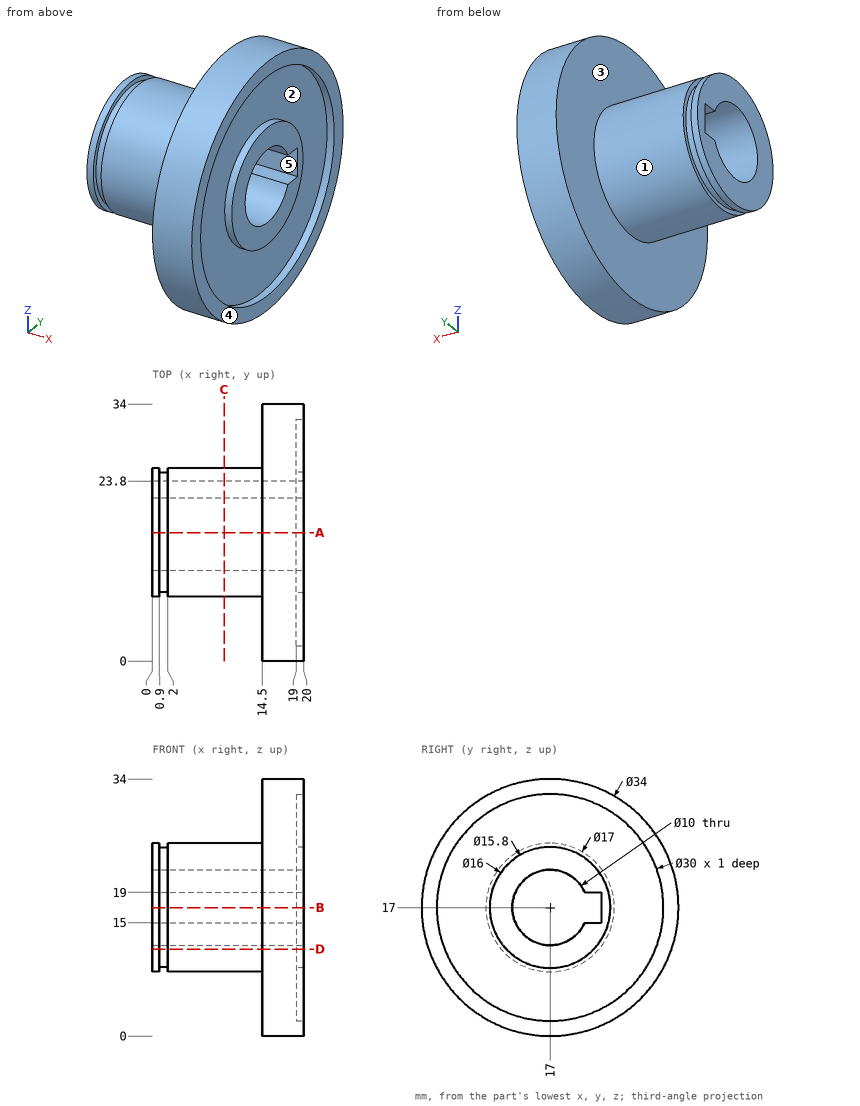
Could you check a few things on this drawing? It's one solid part, dimensions in mm from its lowest x, y, z. A direction names the side the tool comes from. Coordinates: 2 decimals unless noted, no trailing zeros. Order: outer loops, then holes, each group sorted by start corner. A loop starts at its lowest first (then second) coordinate and runs counter-clockwise, first axis right, second up. Notation, with made-up numbers: (-14.5, 0.5) -> (37.5, 0.5) arc R20 cw to (37.5, 20.5) -> close; hole circle Ø10 at (52, 0.25). An arc over 180 degrees is marked (long way). One line per item, written item: value. Start each with the question number.
1) Imagine slicing it at D-D on z = 11.5. List the corners of the cut face in (x, y) for me.
2) We'd pull the mould along Z, two halves only. Please class the marked faces 1, 2 and 3: +Z half, -Z half, draft (parallel to the pull), parting line (faces both ways), or undercut.
3) I'm going to push flat-ended pins straight in: pin 1 (8 mm diameter, centred on y = 17, z = 17, fed in from +X); pin 2 (0.7 mm diameter, centred on x = 7, y = 23, fed in from -Z); pin 3 (13.5 mm diameter, centred on y = 16.5, z = 18, fed in from -X); pin 4 (6 mm diameter, centred on y = 29.5, z = 28.5, fed in from -X). Where does each tip first touch, or does it pass through?
4) If I drill on L1, parallel to Y at x = 19.8, z = 17; L2, parallel to Z at x = 9.5, y = 17; L3, parallel to Y at x = 5, z = 17, over which ranges is the centre line in solid material (lowest first)? Write a range as [from, to].
5) Imagine slicing it at C-C on x = 9.5. List the corners of the cut face in (y, z) for me, plus the area to 3 significant figures.
6) Imagine slicing it at A-A on y = 17. List the corners of the cut face in (x, z) for me.
7) Which directions (+Z, -Z, +X, -X, +Y, -Y) give clear straight access to the entire face, cutting with the end or side of a thin tool? Please do the marked faces 4 and 5.
8) Imagine slicing it at B-B on z = 17. List the corners of the cut face in (x, y) for me.
Answer list:
1. outline: (0, 10.52) -> (0.9, 10.52) -> (0.9, 11.33) -> (2, 11.33) -> (2, 10.52) -> (14.5, 10.52) -> (14.5, 0.91) -> (20, 0.91) -> (20, 3.04) -> (19, 3.04) -> (19, 11.19) -> (20, 11.19) -> (20, 22.81) -> (19, 22.81) -> (19, 30.96) -> (20, 30.96) -> (20, 33.09) -> (14.5, 33.09) -> (14.5, 23.48) -> (2, 23.48) -> (2, 22.67) -> (0.9, 22.67) -> (0.9, 23.48) -> (0, 23.48) -> close
2. face 1: parting line
2. face 2: undercut
2. face 3: draft
3. pin 1: passes through
3. pin 2: stops at z = 10.65
3. pin 3: stops at x = 0
3. pin 4: stops at x = 14.5
4. L1: y = [0, 2], [9, 12], [23.8, 25], [32, 34]
4. L2: z = [8.5, 12], [22, 25.5]
4. L3: y = [8.5, 12], [23.8, 25.5]
5. outline: circle Ø17 at (17, 17); hole (21.58, 15) -> (23.8, 15) -> (23.8, 19) -> (21.58, 19) arc R5 ccw (long way) to start
5. area: 141 mm2
6. outline: (0, 8.5) -> (0.9, 8.5) -> (0.9, 9.1) -> (2, 9.1) -> (2, 8.5) -> (14.5, 8.5) -> (14.5, 0) -> (20, 0) -> (20, 2) -> (19, 2) -> (19, 9) -> (20, 9) -> (20, 12) -> (0, 12) -> close; (0, 22) -> (20, 22) -> (20, 25) -> (19, 25) -> (19, 32) -> (20, 32) -> (20, 34) -> (14.5, 34) -> (14.5, 25.5) -> (2, 25.5) -> (2, 24.9) -> (0.9, 24.9) -> (0.9, 25.5) -> (0, 25.5) -> close
7. face 4: +Z, -Z, +X, +Y, -Y
7. face 5: +X, -X
8. outline: (0, 8.5) -> (0.9, 8.5) -> (0.9, 9.1) -> (2, 9.1) -> (2, 8.5) -> (14.5, 8.5) -> (14.5, 0) -> (20, 0) -> (20, 2) -> (19, 2) -> (19, 9) -> (20, 9) -> (20, 12) -> (0, 12) -> close; (0, 23.8) -> (20, 23.8) -> (20, 25) -> (19, 25) -> (19, 32) -> (20, 32) -> (20, 34) -> (14.5, 34) -> (14.5, 25.5) -> (2, 25.5) -> (2, 24.9) -> (0.9, 24.9) -> (0.9, 25.5) -> (0, 25.5) -> close
